CAD build for the part. Positions are in the model's coordinates, mm. Round coordinates to 2 decimals unless told otherwise and drop trailing zeros. Loops run counter-clockwise (first coordinate to the right, second up) from the corner with the lowest first, then second, coordinate; pieces in that order, holes last.
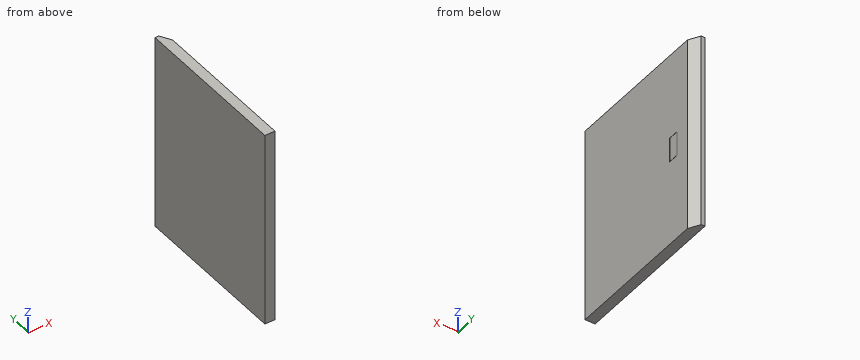
```python
from build123d import *

# Parameters (mm, degrees)
BOSS_EXTRUDE1_DEPTH     = 780
SKETCH2_W               = 98.4
SKETCH2_H               = 42.4
SKETCH2_W_2             = 96
SKETCH2_H_2             = 40
CUT_EXTRUDE_THIN1_DEPTH = 2


with BuildPart() as part:
    # Sketch1 → Boss-Extrude1 (new body)
    with BuildSketch(Plane.XY):
        Polygon((0, 0), (0, -630), (40, -630), (40, -43.301270189), (15, 0), align=None)
    extrude(amount=BOSS_EXTRUDE1_DEPTH)

    # Sketch2 → Cut-Extrude-Thin1 (cut)
    with BuildSketch(Plane(origin=(40, 0, 0), x_dir=(0, 0, -1), z_dir=(1, 0, 0))):
        with Locations((-390, -123.301270189)):
            Rectangle(SKETCH2_W, SKETCH2_H)
        with Locations((-390, -123.301270189)):
            Rectangle(SKETCH2_W_2, SKETCH2_H_2, mode=Mode.SUBTRACT)
    extrude(amount=-CUT_EXTRUDE_THIN1_DEPTH, mode=Mode.SUBTRACT)


solid = part.part
```
Item 1: Flat gauge pins, fed straight in: P1, Ø2, axis at x = 13.5, y = -116.5, coming from the -Z side; P2, Ø0.6, axis at x = 39, z = 408, coming from the +Y side; P3, Ø1.6, axis at x = 39, z = 411, coming from the +Y side; P4, Ø6, axis at x = 20, z = 567.5, coming from the +Y side. Where does each tip first touch, or does it go through?
Answers follow:
P1: stops at z = 0
P2: stops at y = -41.05
P3: stops at y = -40.18
P4: stops at y = -3.46
Item 2: Cut at A-A, the plane z = 111.5. Give the cut face in (x, y).
Answers follow:
outline: (0, -630) - (40, -630) - (40, -43.3) - (15, 0) - (0, 0) - close
Item 3: Probe line 1 (Y direction, x = 28.5, z = 93); line 2 (Y direction, x = 33, z = 671.5); line 3 (X direction, y = -32, z = 668). List the from-to ranges inside material, lowest first.
Answers follow:
line 1: y = -630 to -23.38
line 2: y = -630 to -31.18
line 3: x = 0 to 33.48
Item 4: Cut at B-B, the plane x = 25.5. Give the cut face in (y, z).
Answers follow:
outline: (-630, 0) - (-18.19, 0) - (-18.19, 780) - (-630, 780) - close
